Source: CAD feature listing. Evaluate the final solid. Frame: model axes, mm. Give positions to 0.01 mm unless a question says otherwise; leave off trailing zeros. Write each loop counter-clockwise with the first axis right and the second up, starting at its lowest first coordinate (ties: lowest second). Pieces come first, ordered by that corner, then holes. Notation, with made-up numbers: (-9.75, 74.25) -> (49.25, 74.25) arc R8 cw to (49.25, 85.25) -> close; hole circle Ø9 at (86.5, 61.5). An arc over 180 degrees is marked (long way). Use one line per item in the form item = value. Start each with the question number.
(1) Cut plane D-D, the plane z = 7. Output: boundary loops of the cut face in (x, y), and give its area (3 significant figures).
(2) Cut plane C-C, the plane x = 2050. Output: boundary loops of the cut face in (y, z), and give its area (3 significant figures).
(3) Cut plane B-B, the plane x = 205. Output: boundary loops of the cut face in (y, z).
(4) First-contact query: P1, Ø10, axis at x = 1644.5, z = 3, coming from the +Y side; P2, Ø12, axis at x = 931.5, z = 12, coming from the +Y side; P3, Ø12.5, axis at x = 1100, z = 11, coming from the +Y side. Flat tips, straight axial feed; report the tip coordinate or a pass-through.
(5) Material intervals for line 1 along X through (y, z) = (434, 10.25); line 2 along Y through (x, z) = (2050, 20); line 3 along Y through (x, z) = (2305, 13), sorted ascending. Write a range as from..to.
(6) Cut plane A-A, the plane y = 151.5. Output: boundary loops of the cut face in (x, z), and give its area (3 significant figures).
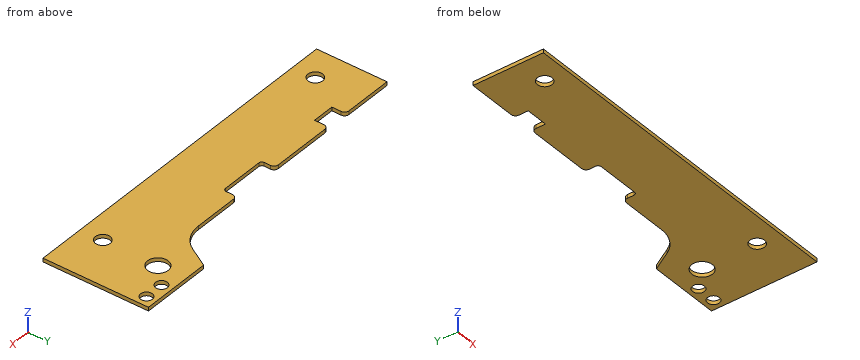
from build123d import *

# Parameters (mm, degrees)
SKETCH1_R           = 50
SKETCH1_R_2         = 70
SKETCH1_R_3         = 40
BOSS_EXTRUDE1_DEPTH = 25


with BuildPart() as part:
    # Sketch1 → Boss-Extrude1 (new body)
    with BuildSketch(Plane.XY):
        with BuildLine():
            Line((0, 0), (0, 477))
            Line((0, 477), (330, 477))
            ThreePointArc((330, 477), (351.213203436, 468.213203436), (360, 447))
            Line((360, 447), (360, 384))
            Line((360, 384), (510, 384))
            Line((510, 384), (510, 447))
            ThreePointArc((510, 447), (518.786796564, 468.213203436), (540, 477))
            Line((540, 477), (943, 477))
            ThreePointArc((943, 477), (964.213203436, 468.213203436), (973, 447))
            Line((973, 447), (973, 404))
            ThreePointArc((973, 404), (978.857864376, 389.857864376), (993, 384))
            Line((993, 384), (1283, 384))
            ThreePointArc((1283, 384), (1297.142135624, 389.857864376), (1303, 404))
            Line((1303, 404), (1303, 447))
            ThreePointArc((1303, 447), (1311.786796564, 468.213203436), (1333, 477))
            Line((1333, 477), (1638.413104807, 477))
            ThreePointArc((1638.413104807, 477), (1742.913104807, 505.000690609), (1819.412414198, 581.5))
            Line((1819.412414198, 581.5), (1896.2, 714.5))
            Line((1896.2, 714.5), (2375, 714.5))
            Line((2375, 714.5), (2375, 0))
            Line((2375, 0), (0, 0))
        make_face()
        with Locations((205, 151.5)):
            Circle(SKETCH1_R, mode=Mode.SUBTRACT)
        with Locations((2050, 151.5)):
            Circle(SKETCH1_R, mode=Mode.SUBTRACT)
        with Locations((2050, 524.5)):
            Circle(SKETCH1_R_2, mode=Mode.SUBTRACT)
        with Locations((2305, 646.5)):
            Circle(SKETCH1_R_3, mode=Mode.SUBTRACT)
        with Locations((2175, 646.5)):
            Circle(SKETCH1_R_3, mode=Mode.SUBTRACT)
    extrude(amount=BOSS_EXTRUDE1_DEPTH)


solid = part.part
Geometry says:
q1.outline = (0, 0) -> (2375, 0) -> (2375, 714.5) -> (1896.2, 714.5) -> (1819.41, 581.5) arc R209 cw to (1638.41, 477) -> (1333, 477) arc R30 ccw to (1303, 447) -> (1303, 404) arc R20 cw to (1283, 384) -> (993, 384) arc R20 cw to (973, 404) -> (973, 447) arc R30 ccw to (943, 477) -> (540, 477) arc R30 ccw to (510, 447) -> (510, 384) -> (360, 384) -> (360, 447) arc R30 ccw to (330, 477) -> (0, 477) -> close; hole circle Ø100 at (205, 151.5); hole circle Ø140 at (2050, 524.5); hole circle Ø100 at (2050, 151.5); hole circle Ø80 at (2175, 646.5); hole circle Ø80 at (2305, 646.5)
q1.area = 1,180,000 mm^2
q2.outline = (0, 0) -> (101.5, 0) -> (101.5, 25) -> (0, 25) -> close; (201.5, 0) -> (454.5, 0) -> (454.5, 25) -> (201.5, 25) -> close; (594.5, 0) -> (714.5, 0) -> (714.5, 25) -> (594.5, 25) -> close
q2.area = 11,900 mm^2
q3.outline = (0, 0) -> (101.5, 0) -> (101.5, 25) -> (0, 25) -> close; (201.5, 0) -> (477, 0) -> (477, 25) -> (201.5, 25) -> close
q4.P1 = 477.29
q4.P2 = 477
q4.P3 = 384
q5.line_1 = 0..360, 510..973, 1303..2375
q5.line_2 = 0..101.5, 201.5..454.5, 594.5..714.5
q5.line_3 = 0..606.5, 686.5..714.5
q6.outline = (0, 0) -> (155, 0) -> (155, 25) -> (0, 25) -> close; (255, 0) -> (2000, 0) -> (2000, 25) -> (255, 25) -> close; (2100, 0) -> (2375, 0) -> (2375, 25) -> (2100, 25) -> close
q6.area = 54,400 mm^2
